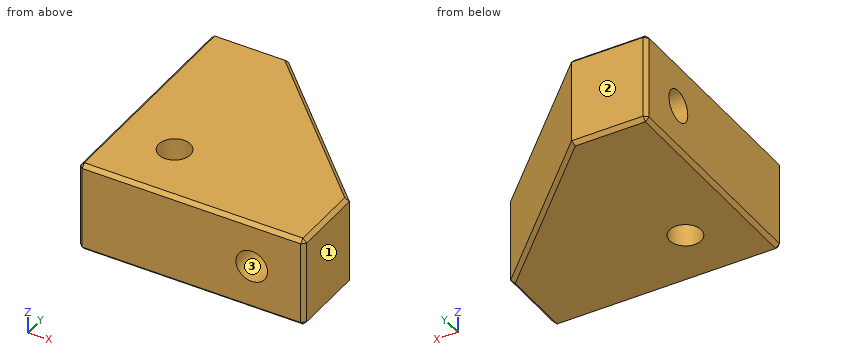
```python
from build123d import *

# Parameters (mm, degrees)
SKETCH_1_W             = 30
SKETCH_1_H             = 30
EXTRUDE_1_DEPTH        = 12
CHAMFER_1_SIZE         = 20
HOLE_WIZARD_M5_1_D     = 4.2
HOLE_WIZARD_M5_2_D     = 4.2
HOLE_WIZARD_M5_2_DEPTH = 12.4
HOLE_WIZARD_M5_2_TIP   = 1.2618073
HOLE_WIZARD_M5_3_D     = 4.2
HOLE_WIZARD_M5_3_DEPTH = 12.4
HOLE_WIZARD_M5_3_TIP   = 1.2618073
CHAMFER_2_SIZE         = 0.5


with BuildPart() as part:
    # 草图1 → 凸台-拉伸1 (new body)
    with BuildSketch(Plane.XY):
        Rectangle(SKETCH_1_W, SKETCH_1_H)
    extrude(amount=EXTRUDE_1_DEPTH)

    # 倒角1
    chamfer_1_edges = [part.edges().sort_by_distance(p)[0] for p in [
        (15, 15, 6),
    ]]
    chamfer(chamfer_1_edges, length=CHAMFER_1_SIZE)

    # M5 螺纹孔1 (through all)
    with Locations(Plane.XY.offset(12)):
        with Locations((-7, -7)):
            Hole(HOLE_WIZARD_M5_1_D / 2)

    # M5 螺纹孔2
    with Locations(Plane(origin=(0, -15, 0), x_dir=(-1, 0, 0), z_dir=(0, -1, 0))):
        with Locations((-8, -6)):
            Hole(HOLE_WIZARD_M5_2_D / 2, depth=HOLE_WIZARD_M5_2_DEPTH)
            with Locations((0, 0, -(HOLE_WIZARD_M5_2_DEPTH + HOLE_WIZARD_M5_2_TIP / 2))):  # 118° drill point
                Cone(0, HOLE_WIZARD_M5_2_D / 2, HOLE_WIZARD_M5_2_TIP, mode=Mode.SUBTRACT)

    # M5 螺纹孔3
    with Locations(Plane.ZY.offset(15)):
        with Locations((6, 8)):
            Hole(HOLE_WIZARD_M5_3_D / 2, depth=HOLE_WIZARD_M5_3_DEPTH)
            with Locations((0, 0, -(HOLE_WIZARD_M5_3_DEPTH + HOLE_WIZARD_M5_3_TIP / 2))):  # 118° drill point
                Cone(0, HOLE_WIZARD_M5_3_D / 2, HOLE_WIZARD_M5_3_TIP, mode=Mode.SUBTRACT)

    # 倒角2
    chamfer_2_edges = [part.edges().sort_by_distance(p)[0] for p in [
        (-15, 0, 12),
        (-10, 15, 0),
        (-10, 15, 12),
        (5, 5, 0),
        (5, 5, 12),
        (0, -15, 12),
        (15, -10, 12),
        (0, -15, 0),
        (-15, 0, 0),
        (15, -10, 0),
        (15, -15, 6),
        (-15, -15, 6),
        (-15, 15, 6),
    ]]
    chamfer(chamfer_2_edges, length=CHAMFER_2_SIZE)


solid = part.part
```
Check sheet for the modelled part. Datum: model origin and axes. Units: mm. Face numbers are marked on the shaded views. Give positions to 0.01 mm unless a question says otherwise; leave off trailing zeros. Loops run counter-clockwise (first coordinate to the right, second up) from the corner with the lowest first, then second, coordinate; pieces in that order, holes last. Notation, with made-up numbers: M 27.5,40 L 54.5,40 A17 cw 54.5,50 Z; hole C 81,5 d6. An arc over 180 degrees is marked long. Answer as CSV lines item,"result".
Item 1: Depth check by flat-ended pin: pin 1 Ø4 at (y, z) = (12, 9) entering from +X; pin 2 Ø1.5 at (y, z) = (8.5, 10) entering from +X; pin 3 Ø3.5 at (x, z) = (8, 6) entering from -Y. Enter the tip coordinate at first touch or a pass-through.
Reply:
pin 1,"x = 0"
pin 2,"x = 2.25"
pin 3,"y = -2.39"
Item 2: Scan lines: L1, parallel to Y at x = -8.5, z = 7.75; L2, parallel to Y at x = -11, z = 6; L3, parallel to Z at x = 8, y = -8.25. Record each from-to range of solid material in increasing order.
Reply:
L1,"-15 to -8.47, -5.53 to 6.84, 9.16 to 15"
L2,"-15 to 5.9, 10.1 to 15"
L3,"0 to 3.9, 8.1 to 12"
Item 3: Sectioned sample at D-D, the plane y = -3. Enter the section's corners in (x, z), then the cut area to 3 significant figures.
Reply:
outline,"M -15,0.5 L -14.5,0 L 12.29,0 L 13,0.5 L 13,11.5 L 12.29,12 L -14.5,12 L -15,11.5 Z; hole C 8,6 d4.2"
area,"322 mm^2"
Item 4: Draft check along X on the marked faces 1, 2 and 3. Enter one of: pulls with the +X half, pulls with the -X half, needs draft (parallel to the pull), parting line crosses it, or undercut.
Reply:
face 1,"pulls with the +X half"
face 2,"needs draft"
face 3,"undercut"
Item 5: Sectioned sample at A-A, the plane y = -7. Enter the section's corners in (x, z).
Reply:
outline,"M -15,0.5 L -14.5,0 L -9.1,0 L -9.1,12 L -14.5,12 L -15,11.5 Z; M -4.9,0 L 14.5,0 L 15,0.5 L 15,11.5 L 14.5,12 L -4.9,12 Z; hole C 8,6 d4.2"
Item 6: Sectioned sample at C-C, the plane z = 11. Enter the section's corners in (x, y).
Reply:
outline,"M -15,-14.5 L -14.5,-15 L 14.5,-15 L 15,-14.5 L 15,-5 L -5,15 L -14.5,15 L -15,14.5 Z; hole C -7,-7 d4.2"
